from build123d import *

# Parameters (mm, degrees)
SKETCH1_W           = 340
SKETCH1_H           = 340
BOSS_EXTRUDE1_DEPTH = 150
SHELL1_T            = -1.5
SKETCH2_W           = 340
SKETCH2_H           = 340
BOSS_EXTRUDE2_DEPTH = 1
SKETCH3_W           = 320
SKETCH3_H           = 320
SKETCH3_W_2         = 316
SKETCH3_H_2         = 316
SKETCH3_R           = 11.25
SKETCH3_W_3         = 24
SKETCH3_H_3         = 80
SKETCH3_W_4         = 45
SKETCH3_H_4         = 45
CUT_EXTRUDE1_DEPTH  = 0.5


with BuildPart() as part:
    # Sketch1 → Boss-Extrude1 (new body)
    with BuildSketch(Plane.XY):
        with Locations((170, 170)):
            Rectangle(SKETCH1_W, SKETCH1_H)
    extrude(amount=BOSS_EXTRUDE1_DEPTH)

    # Shell1
    shell1_openings = [part.faces().sort_by_distance(p)[0] for p in [
        (170, 170, 150),
    ]]
    offset(amount=SHELL1_T, openings=shell1_openings, kind=Kind.INTERSECTION)

    # Sketch2 → Boss-Extrude2 (add)
    with BuildSketch(Plane.XY.offset(150)):
        with Locations((170, 170)):
            Rectangle(SKETCH2_W, SKETCH2_H)
    extrude(amount=BOSS_EXTRUDE2_DEPTH)

    # Sketch3 → Cut-Extrude1 (cut)
    # profile 1 of 5: a face of its own
    with BuildSketch(Plane.XY.offset(151)):
        with Locations((170, 170)):
            Rectangle(SKETCH3_W, SKETCH3_H)
        with Locations((170, 170)):
            Rectangle(SKETCH3_W_2, SKETCH3_H_2, mode=Mode.SUBTRACT)
    # profile 2 of 5: a face of its own
    with BuildSketch(Plane.XY.offset(151)):
        with Locations((170, 207.5)):
            Circle(SKETCH3_R)
    # profile 3 of 5: a face of its own
    with BuildSketch(Plane.XY.offset(151)):
        with Locations((170, 127.5)):
            Circle(SKETCH3_R)
    # profile 4 of 5: a face of its own
    with BuildSketch(Plane.XY.offset(151)):
        with Locations((39, 170)):
            Rectangle(SKETCH3_W_3, SKETCH3_H_3)
    # profile 5 of 5: a face of its own
    with BuildSketch(Plane.XY.offset(151)):
        with Locations((170, 285.5)):
            Rectangle(SKETCH3_W_4, SKETCH3_H_4)
    extrude(amount=-CUT_EXTRUDE1_DEPTH, mode=Mode.SUBTRACT)


solid = part.part
Here's how the part is built. I have some questions about the finished solid (model axes, mm). A direction names the side the tool comes from. Coordinates: 2 decimals unless noted, no trailing zeros. Write each loop counter-clockwise with the first axis right and the second up, starting at its lowest first coordinate (ties: lowest second). Pieces come first, ordered by that corner, then holes. Notation, with made-up numbers: (18.25, 7.5) - (38.25, 7.5) arc R15 cw to (38.25, 28.5) - close; hole circle Ø8 at (-31, -1). An arc over 180 degrees is marked (long way). Use one line per item in the form item = value.
1) Suppose I cut it at B-B, the plane y = 316.5. Write out the boundary of the cut face in (x, z), plus the area to 3 significant figures.
Solved:
outline = (0, 0) - (340, 0) - (340, 151) - (330, 151) - (330, 150.5) - (328, 150.5) - (328, 151) - (12, 151) - (12, 150.5) - (10, 150.5) - (10, 151) - (0, 151) - close; hole (1.5, 1.5) - (338.5, 1.5) - (338.5, 150) - (1.5, 150) - close
area = 1,290 mm2
2) Suppose I cut it at A-A, the plane x = 170. Write out the boundary of the cut face in (y, z), plus the area to 3 significant figures.
Solved:
outline = (0, 0) - (340, 0) - (340, 151) - (330, 151) - (330, 150.5) - (328, 150.5) - (328, 151) - (308, 151) - (308, 150.5) - (263, 150.5) - (263, 151) - (218.75, 151) - (218.75, 150.5) - (196.25, 150.5) - (196.25, 151) - (138.75, 151) - (138.75, 150.5) - (116.25, 150.5) - (116.25, 151) - (12, 151) - (12, 150.5) - (10, 150.5) - (10, 151) - (0, 151) - close; hole (1.5, 1.5) - (338.5, 1.5) - (338.5, 150) - (1.5, 150) - close
area = 1,250 mm2
3) Suppose I cut it at C-C, the plane z = 86.5. Write out the boundary of the cut face in (x, y), plus the area to 3 significant figures.
Solved:
outline = (0, 0) - (340, 0) - (340, 340) - (0, 340) - close; hole (1.5, 1.5) - (338.5, 1.5) - (338.5, 338.5) - (1.5, 338.5) - close
area = 2,030 mm2
4) On a 3-axis mill with a long thin cutter (end or side, diameter ignored), from which of +Z, -Z, +X, -X, +Y, -Y can I reach the whole of each face in a straight line? I mean faces 4 (the flat face through (1.5, 168, 75)), 5 (the flat face through (168, 0, 74)), 6 (the cylindrical face through (180.73, 210.88, 150.75)). Say none if no direction works.
Solved:
face_4 = none
face_5 = +Z, -Z, +X, -X, -Y
face_6 = +Z
5) I'm going to push a flat-ended pin straight in: P1, Ø22.5, axis at x = 170.5, y = 285.5, coming from the +Z side. Where does the tip first touch, or does it pass through?
Solved:
P1 = 150.5
6) Thinking about a two-plate mould opening in Z: for faces 1 (the flat face through (168, 338.5, 75)), 2 (the cylindrical face through (180.73, 130.88, 150.75)), 3 (the flat face through (168, 172, 151)), which applies, released by +Z, released by -Z, zero draft, split by the parting line, or undercut?
Solved:
face_1 = undercut
face_2 = zero draft
face_3 = released by +Z
7) I need wall thicknesses on line 1 (Y direction, x = 170, z = 150.7); line 2 (Z direction, x = 22, y = 215.5); line 3 (Y direction, x = 80.5, z = 44). Which ranges of each line are inside material? Lowest first, please.
Solved:
line_1 = 0 to 10, 12 to 116.25, 138.75 to 196.25, 218.75 to 263, 308 to 328, 330 to 340
line_2 = 0 to 1.5, 150 to 151
line_3 = 0 to 1.5, 338.5 to 340
